For this review, take the finished solid that the model builds, in its own axes (mm). Coordinates: 2 decimals unless noted, no trailing zeros. Loops run counter-clockwise (first coordinate to the right, second up) from the corner with the lowest first, then second, coordinate; pieces in that order, holes last.
1. Mouldability with a two-part tool opening along X and no side actions: class faces 1 (the face through (-9.15, 0.07, 4.06)), 2 (the face through (-7, 5, 4)), 3 (the face through (-17, 0, 4)), 4 (the face through (3, 0, 4)) as pulls with the +X half, pulls with the -X half, needs draft (parallel to the pull), parting line crosses it, or undercut.
2. Take a section at B-B, the plane x = -7.5. State the section outline as (y, z) points.
3. Take a section at D-D, the plane z = 5.5. State the section outline as (x, y) points, then the cut area to 3 significant figures.
4. To check wall thickness, follow probe 1 along Y at (x, z) = (-7.5, 3.25); probe 2 along X at (y, z) = (-2.85, 4); probe 3 along Z at (x, y) = (0, 4.1). State the ranges of each line that lie inside material, in increasing order.
5. Take a section at C-C, the plane y = 0. State the section outline as (x, z) points.
6. Take a section at A-A, the plane z = 4. State the section outline as (x, y) points.
```python
from build123d import *

# Parameters (mm, degrees)
SKETCH_1_W                  = 20
SKETCH_1_H                  = 10
SKETCH_1_R                  = 2
EXTRUDE_1_DEPTH             = 8
SKETCH_2_W                  = 9.758246521
SKETCH_2_H                  = 16.171909484
CUT_EXTRUDE_1_DEPTH         = 22
MOVE_FACE_1_BY              = 7
HOLE_WIZARD_3_3_3_3_1_D     = 3.3
HOLE_WIZARD_3_3_3_3_1_DEPTH = 11.5
HOLE_WIZARD_3_3_3_3_1_TIP   = 0.991420021
HOLE_WIZARD_M3_1_D          = 2.5


with BuildPart() as part:
    # 草图1 → 凸台-拉伸1 (new body)
    with BuildSketch(Plane.XY):
        Rectangle(SKETCH_1_W, SKETCH_1_H)
        Circle(SKETCH_1_R, mode=Mode.SUBTRACT)
    extrude(amount=EXTRUDE_1_DEPTH)

    # 草图2 → 切除-拉伸1 (cut)
    with BuildSketch(Plane(origin=(0, 0, 0), x_dir=(-1, 0, 0), z_dir=(0, 0, -1))):
        with Locations((-7.879123261, 2.238600796)):
            Rectangle(SKETCH_2_W, SKETCH_2_H)
    extrude(amount=-CUT_EXTRUDE_1_DEPTH, mode=Mode.SUBTRACT)

    # Move Face 1: a face moved outward by 7.0
    extrude(part.faces().sort_by_distance((-10, 0, 4))[0], amount=MOVE_FACE_1_BY, dir=(-1, 0, 0))

    # Ø3.3 (3.3) 直径孔1
    with Locations(Plane(origin=(0, 0, 0), x_dir=(-1, 0, 0), z_dir=(0, 0, -1))):
        with Locations((7.5, 0), (14, 0)):
            Hole(HOLE_WIZARD_3_3_3_3_1_D / 2, depth=HOLE_WIZARD_3_3_3_3_1_DEPTH)
            with Locations((0, 0, -(HOLE_WIZARD_3_3_3_3_1_DEPTH + HOLE_WIZARD_3_3_3_3_1_TIP / 2))):  # 118° drill point
                Cone(0, HOLE_WIZARD_3_3_3_3_1_D / 2, HOLE_WIZARD_3_3_3_3_1_TIP, mode=Mode.SUBTRACT)

    # M3 螺纹孔1 (through all)
    with Locations(Plane(origin=(0, 5, 0), x_dir=(1, 0, 0), z_dir=(0, 1, 0))):
        with Locations((0, -4)):
            Hole(HOLE_WIZARD_M3_1_D / 2)


solid = part.part
```
Results list:
1. face 1: undercut
1. face 2: needs draft
1. face 3: pulls with the -X half
1. face 4: pulls with the +X half
2. outline: (-5, 0) - (-1.65, 0) - (-1.65, 8) - (-5, 8) - close; (1.65, 0) - (5, 0) - (5, 8) - (1.65, 8) - close
3. outline: (-17, -5) - (3, -5) - (3, 5) - (-17, 5) - close; hole circle Ø3.3 at (-14, 0); hole circle Ø3.3 at (-7.5, 0); hole circle Ø4 at (0, 0)
3. area: 170 mm2
4. probe 1: y = -5 to -1.65, 1.65 to 5
4. probe 2: x = -17 to -1.25, 1.25 to 3
4. probe 3: z = 0 to 2.75, 5.25 to 8
5. outline: (-17, 0) - (-15.65, 0) - (-15.65, 8) - (-17, 8) - close; (-12.35, 0) - (-9.15, 0) - (-9.15, 8) - (-12.35, 8) - close; (-5.85, 0) - (-2, 0) - (-2, 8) - (-5.85, 8) - close; (2, 0) - (3, 0) - (3, 8) - (2, 8) - close
6. outline: (-17, -5) - (-1.25, -5) - (-1.25, -1.56) arc R2 cw to (-1.25, 1.56) - (-1.25, 5) - (-17, 5) - close; (1.25, -5) - (3, -5) - (3, 5) - (1.25, 5) - (1.25, 1.56) arc R2 cw to (1.25, -1.56) - close; hole circle Ø3.3 at (-14, 0); hole circle Ø3.3 at (-7.5, 0)
